Here's how the part is built. I have some questions about the finished solid (model axes, mm). A direction names the side the tool comes from. Round coordinates to 2 decimals unless told otherwise and drop trailing zeros. Order: outer loops, then holes, each group sorted by start corner. A loop starts at its lowest first (then second) coordinate and runs counter-clockwise, first axis right, second up. Notation, with made-up numbers: (6.25, -14) -> (21.25, -14) arc R27 cw to (21.25, 6) -> close; hole circle Ø9 at (70, 18.5). An arc over 180 degrees is marked (long way). Answer in a Markdown table with one row per item.
```python
from build123d import *

# Parameters (mm, degrees)
SKETCH1_W             = 120
SKETCH1_H             = 90
SKETCH1_R             = 40
BOSS_EXTRUDE1_DEPTH   = 8
SKETCH3_W             = 8
SKETCH3_H             = 90
BOSS_EXTRUDE2_DEPTH   = 50
SKETCH4_W             = 8
SKETCH4_H             = 90
BOSS_EXTRUDE3_DEPTH   = 100
SKETCH5_W             = 178.684775764
SKETCH5_H             = 148.432517326
CUT_EXTRUDE1_DEPTH    = 156.32224567
SKETCH6_W             = 8
SKETCH6_H             = 90
BOSS_EXTRUDE4_DEPTH   = 55
SKETCH7_R             = 3.03642696
SKETCH7_R_2           = 2.873850802
SKETCH7_R_3           = 2.874430555
SKETCH7_R_4           = 2.981394427
SKETCH7_R_5           = 24.990861791
CUT_EXTRUDE2_DEPTH    = 35
M4_TAPPED_HOLE1_D     = 3.3
M4_TAPPED_HOLE1_DEPTH = 10.1
M4_TAPPED_HOLE1_TIP   = 0.991420021


with BuildPart() as part:
    # Sketch1 → Boss-Extrude1 (new body)
    with BuildSketch(Plane.XY):
        Rectangle(SKETCH1_W, SKETCH1_H)
        Circle(SKETCH1_R, mode=Mode.SUBTRACT)
    extrude(amount=BOSS_EXTRUDE1_DEPTH)

    # Sketch3 → Boss-Extrude2 (add)
    with BuildSketch(Plane.ZY.offset(60)):
        with Locations((4, 0)):
            Rectangle(SKETCH3_W, SKETCH3_H)
    extrude(amount=BOSS_EXTRUDE2_DEPTH)

    # Sketch4 → Boss-Extrude3 (add)
    with BuildSketch(Plane.XY.offset(8)):
        with Locations((-66, 0)):
            Rectangle(SKETCH4_W, SKETCH4_H)
    extrude(amount=BOSS_EXTRUDE3_DEPTH)

    # Sketch5 → Cut-Extrude1 (cut, through all)
    with BuildSketch(Plane.XY.offset(8)):
        with Locations((27.342387882, -29.216258663)):
            Rectangle(SKETCH5_W, SKETCH5_H)
    extrude(amount=-CUT_EXTRUDE1_DEPTH, mode=Mode.SUBTRACT)

    # Sketch6 → Boss-Extrude4 (add)
    with BuildSketch(Plane(origin=(0, 0, 0), x_dir=(-1, 0, 0), z_dir=(0, 0, -1))):
        with Locations((66, 0)):
            Rectangle(SKETCH6_W, SKETCH6_H)
    extrude(amount=BOSS_EXTRUDE4_DEPTH)

    # Sketch7 → Cut-Extrude2 (cut)
    with BuildSketch(Plane.ZY.offset(70)):
        with Locations(Location((-49.227416998, 22.627416998, 0), (0, 0, 270))):
            Circle(SKETCH7_R)
        with Locations(Location((-49.227416998, -22.627416998, 0), (0, 0, 270))):
            Circle(SKETCH7_R_2)
        with Locations(Location((-3.972583002, -22.627416998, 0), (0, 0, 270))):
            Circle(SKETCH7_R_3)
        with Locations(Location((-3.972583002, 22.627416998, 0), (0, 0, 270))):
            Circle(SKETCH7_R_4)
        with Locations(Location((-26.59999988, 0.009138209, 0), (0, 0, 270))):
            Circle(SKETCH7_R_5)
    extrude(amount=-CUT_EXTRUDE2_DEPTH, mode=Mode.SUBTRACT)

    # M4 Tapped Hole1
    with Locations(Plane.ZY.offset(70)):
        with Locations((101, 0), (101, -10)):
            Hole(M4_TAPPED_HOLE1_D / 2, depth=M4_TAPPED_HOLE1_DEPTH)
            with Locations((0, 0, -(M4_TAPPED_HOLE1_DEPTH + M4_TAPPED_HOLE1_TIP / 2))):  # 118° drill point
                Cone(0, M4_TAPPED_HOLE1_D / 2, M4_TAPPED_HOLE1_TIP, mode=Mode.SUBTRACT)


solid = part.part
```
1. Please list where these lines run through material, in increasing order: line 1 along X through (y, z) = (-21, 37.5); line 2 along Z through (x, y) = (-73, 9.5); line 3 along Z through (x, y) = (-66, -3.5).
Numbers:
| item | result |
|---|---|
| line 1 | x = -70 to -62 |
| line 2 | z = 0 to 8 |
| line 3 | z = -55 to -51.34, -1.86 to 108 |
2. Suppose I cut it at A-A on z = 101. Write out the boundary of the cut face in (x, y).
Numbers:
| item | result |
|---|---|
| outline | (-70, -45) -> (-62, -45) -> (-62, -11.65) -> (-70, -11.65) -> close; (-70, -8.35) -> (-62, -8.35) -> (-62, -1.65) -> (-70, -1.65) -> close; (-70, 1.65) -> (-62, 1.65) -> (-62, 45) -> (-70, 45) -> close |
3. For pin 1 Ø8 at (x, y) = (-98, 18.5) entering from +Z; pin 2 Ø6.5 at (y, z) = (-22.63, -49.23) entering from -X, each with a flat end and sliding along its axis, tell me the tip position at first contact or that it passes through.
Numbers:
| item | result |
|---|---|
| pin 1 | stops at z = 8 |
| pin 2 | stops at x = -70 |
4. Suppose I cut it at D-D on y = 39. Write out the boundary of the cut face in (x, z).
Numbers:
| item | result |
|---|---|
| outline | (-110, 0) -> (-70, 0) -> (-70, -55) -> (-62, -55) -> (-62, 108) -> (-70, 108) -> (-70, 8) -> (-110, 8) -> close |
5. Suppose I cut it at B-B on y = 0. Write out the boundary of the cut face in (x, z).
Numbers:
| item | result |
|---|---|
| outline | (-110, 0) -> (-70, 0) -> (-70, -1.61) -> (-62, -1.61) -> (-62, 99.35) -> (-70, 99.35) -> (-70, 8) -> (-110, 8) -> close; (-70, -55) -> (-62, -55) -> (-62, -51.59) -> (-70, -51.59) -> close; (-70, 102.65) -> (-62, 102.65) -> (-62, 108) -> (-70, 108) -> close |
6. For faces 1 (the face through (-65.94, -9.93, 102.65)), 2 (the face through (-70, 9, -52)), 3 (the face through (-90, -1, 8)), which set-ups out of +Z, -Z, +X, -X, +Y, -Y let a thin tool reach every point of the face, with its end or its side?
Numbers:
| item | result |
|---|---|
| face 1 | +X, -X |
| face 2 | -Z, -X, +Y, -Y |
| face 3 | +Z, -X, +Y, -Y |
7. We'd pull the mould along Y, two halves only. Please class faces 4 (the face through (-68, 45, 27)), 5 (the face through (-90, -1, 0)), 6 (the face through (-66.06, -25.37, -3.11)): released by +Y, released by -Y, zero draft, split by the parting line, or undercut.
Numbers:
| item | result |
|---|---|
| face 4 | released by +Y |
| face 5 | zero draft |
| face 6 | undercut |
8. Suppose I cut it at C-C on z = -26.6. Write out the boundary of the cut face in (x, y), then the cut area to 3 significant figures.
Numbers:
| item | result |
|---|---|
| outline | (-70, -45) -> (-62, -45) -> (-62, -24.98) -> (-70, -24.98) -> close; (-70, 25) -> (-62, 25) -> (-62, 45) -> (-70, 45) -> close |
| area | 320 mm2 |
